Source: three-view drawing plus pictorial views. Frame: mm from the lowest corner of the part. A direction names the side the tool comes from. Give positions to 0.01 mm unless a question says otherwise; leave off trailing zeros. Loops run counter-clockwise (first coordinate to the right, second up) from the corner with the lowest first, then second, coordinate; pieces in that order, holes last. Notation, with made-up numbers: (-15, 49.5) - (10, 49.5) arc R33 cw to (10, 88.5) - close; hole circle Ø1 at (58.5, -15.5). An arc over 180 degrees is marked (long way). Put each result on its own line as item: value.
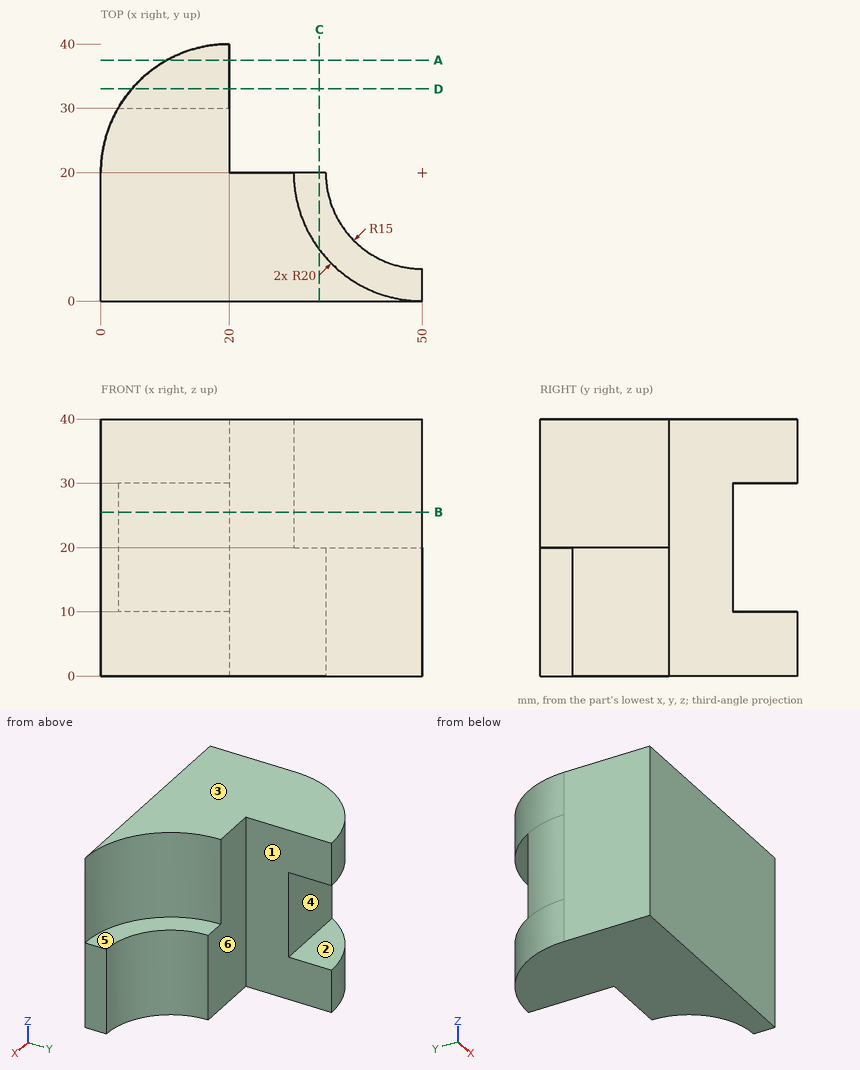
1) Pin query (flat end, axial travel): P1, Ø16.5, axis at x = 29.5, z = 14.5, coming from the +Y side; P2, Ø6, axis at x = 14.5, z = 20, coming from the +Y side; P3, Ø1, axis at y = 12.5, z = 33, coming from the +X side. Return the tip coordinate at first contact, or that it passes through.
Check result:
P1: y = 20
P2: y = 30
P3: x = 31.67
2) Material intervals for line 1 along Z through (x, y) = (4.5, 32); line 2 along Z through (x, y) = (34, 9), sorted ascending. Write a range as [from, to].
Check result:
line 1: [0, 10], [30, 40]
line 2: [0, 20]
3) Mould query, pull axis Z, two halves, no side actions, for the marked faces 1, 2 and 3. Classes: pulls with the +Z half, pulls with the -Z half, needs draft (parallel to the pull), parting line crosses it, or undercut.
Check result:
face 1: needs draft
face 2: undercut
face 3: pulls with the +Z half
4) Section query A-A, the plane y = 37.5. Output: boundary loops of the cut face in (x, z).
Check result:
outline: (10.32, 0) - (20, 0) - (20, 10) - (10.32, 10) - close; (10.32, 30) - (20, 30) - (20, 40) - (10.32, 40) - close
5) Section query D-D, the plane y = 33. Output: boundary loops of the cut face in (x, z), plus the area to 3 significant figures.
Check result:
outline: (4.8, 0) - (20, 0) - (20, 10) - (4.8, 10) - close; (4.8, 30) - (20, 30) - (20, 40) - (4.8, 40) - close
area: 304 mm²
6) Access query for the marked faces 4, 5 and 6. Directions: +Z, -Z, +X, -X, +Y, -Y. A direction counts if a zero-diameter tool reaches every point of the face in a straight line with its end or side. Return the directions, or none.
Check result:
face 4: +X, -X, +Y
face 5: +Z, +X, +Y
face 6: +Z, -Z, +X, +Y
7) Section query C-C, the plane x = 34. Output: boundary loops of the cut face in (y, z), plus the area to 3 significant figures.
Check result:
outline: (0, 0) - (20, 0) - (20, 20) - (8, 20) - (8, 40) - (0, 40) - close
area: 560 mm²
8) Section query B-B, the plane z = 25.5. Output: boundary loops of the cut face in (x, y), plus the area to 3 significant figures.
Check result:
outline: (0, 0) - (50, 0) arc R20 cw to (30, 20) - (20, 20) - (20, 30) - (2.68, 30) arc R20 ccw to (0, 20) - close
area: 877 mm²
